Model file for the job. Use its own axes, mm. A direction names the side the tool comes from. Coordinates: 2 decimals unless noted, no trailing zeros. Loops run counter-clockwise (first coordinate to the right, second up) from the corner with the lowest first, then second, coordinate; pieces in that order, holes last. Notation, with made-up numbers: (-37, -34) -> (17, -34) arc R31 cw to (17, 0) -> close; hole circle Ø11 at (-16, -30.5). An arc over 180 degrees is marked (long way). Use one line per item in the form item = value.
```python
from build123d import *

# Parameters (mm, degrees)
CUT_EXTRUDE1_DEPTH = 1.5
FILLET1_R          = 0.275
CHAMFER1_SIZE      = 0.3
FILLET2_R          = 0.125


with BuildPart() as part:
    # Sketch3 → Revolve1 (revolve)
    with BuildSketch(Plane(origin=(0, 0, 0), x_dir=(0, 0, -1), z_dir=(1, 0, 0)), mode=Mode.PRIVATE) as revolve1_sk:
        Polygon((-3, 0.6), (-3, 2.75), (0, 2.75), (0, 1.5), (5, 1.5), (5, 0.6), align=None)
    revolve(revolve1_sk.sketch.rotate(Axis((0, 0, 3), (0, 0, -1)), 90), axis=Axis((0, 0, 3), (0, 0, -1)))

    # Sketch4 → Cut-Extrude1 (cut)
    with BuildSketch(Plane.XY.offset(3)):
        Polygon((0, 1.443375673), (-1.25, 0.721687836), (-1.25, -0.721687836), (0, -1.443375673), (1.25, -0.721687836), (1.25, 0.721687836), align=None)
    extrude(amount=-CUT_EXTRUDE1_DEPTH, mode=Mode.SUBTRACT)

    # Fillet1
    fillet1_edges = [part.edges().sort_by_distance(p)[0] for p in [
        (-2.75, 0, 3),
    ]]
    fillet(fillet1_edges, radius=FILLET1_R)

    # Chamfer1
    chamfer1_edges = [part.edges().sort_by_distance(p)[0] for p in [
        (-1.5, 0, -5),
    ]]
    chamfer(chamfer1_edges, length=CHAMFER1_SIZE)

    # Cut-Extrude2 cone 1 section (through the dimple's axis) → Cut-Extrude2 (revolve, cut)
    with BuildSketch(Plane(origin=(0, 0, 1.5), x_dir=(0, -1, 0), z_dir=(1, 0, 0))):
        Polygon((0, 0), (1.25, 0), (0, 0.721687836), align=None)
    revolve(axis=Axis((0, 0, 1.5), (0, 0, -1)), mode=Mode.SUBTRACT)

    # Fillet2
    fillet2_edges = [part.edges().sort_by_distance(p)[0] for p in [
        (-1.5, 0, 0),
    ]]
    fillet(fillet2_edges, radius=FILLET2_R)


solid = part.part
```
Q1. Pin check, flat tips, straight feed: pin 1 Ø0.7 at (y, z) = (-0.5, 2.5) entering from +X; pin 2 Ø1.5 at (x, z) = (2, -0.5) entering from +Y; pin 3 Ø0.7 at (y, z) = (0.5, 2) entering from -X. Stop position of each tip, or through.
Result:
pin_1 = 2.75
pin_2 = 2.34
pin_3 = -2.75
Q2. Band-saw the part on A-A, the plane z = 0.75. Write the cut outline in (x, y), and give its area (3 significant figures).
Result:
outline = circle Ø5.5 at (0, 0); hole circle Ø1.2 at (0, 0)
area = 22.6 mm2
Q3. Band-saw the part on B-B, the plane z = -1.75. Write the cut outline in (x, y), and give its area (3 significant figures).
Result:
outline = circle Ø3 at (0, 0); hole circle Ø1.2 at (0, 0)
area = 5.94 mm2
Q4. Wall check: line 1 along X through (y, z) = (-0.05, -1); line 2 along Z through (x, y) = (-1.55, 0.7). Give the ranges that are in metal, low to high.
Result:
line_1 = -1.5 to -0.6, 0.6 to 1.5
line_2 = 0 to 3
Q5. Mould opens along Y. For faces 1 (the face through (1.43, -0.45, -2.44)), 2 (the face through (0.63, 1.08, 2.26)), 3 (the face through (2, 0, 0)) say: released by +Y, released by -Y, zero draft, split by the parting line, or undercut.
Result:
face_1 = split by the parting line
face_2 = undercut
face_3 = zero draft
Q6. Which spindle directions (+Z, -Z, +X, -X, +Y, -Y) get a long thin tool onto all of the face, cutting with end or side? Do faces 4 (the face through (-0.596, 2.685, 1.343)), 5 (the face through (-1.25, 0, 2)). Say none if no direction does.
Result:
face_4 = +Z, -Z
face_5 = +Z
